The drawing under review shows one solid part. Ordinate dimensions are in mm from its lowest x, y, z. Coordinates: 2 decimals unless noted, no trailing zeros. Order: outer loops, then holes, each group sorted by start corner. A loop starts at its lowest first (then second) coordinate and runs counter-clockwise, first axis right, second up. Notation, with made-up numbers: (-30.5, 89.25) -> (23.5, 89.25) arc R22 cw to (23.5, 106.25) -> close; hole circle Ø1 at (17, -21). An arc over 180 degrees is marked (long way). Write item = value, one per line.
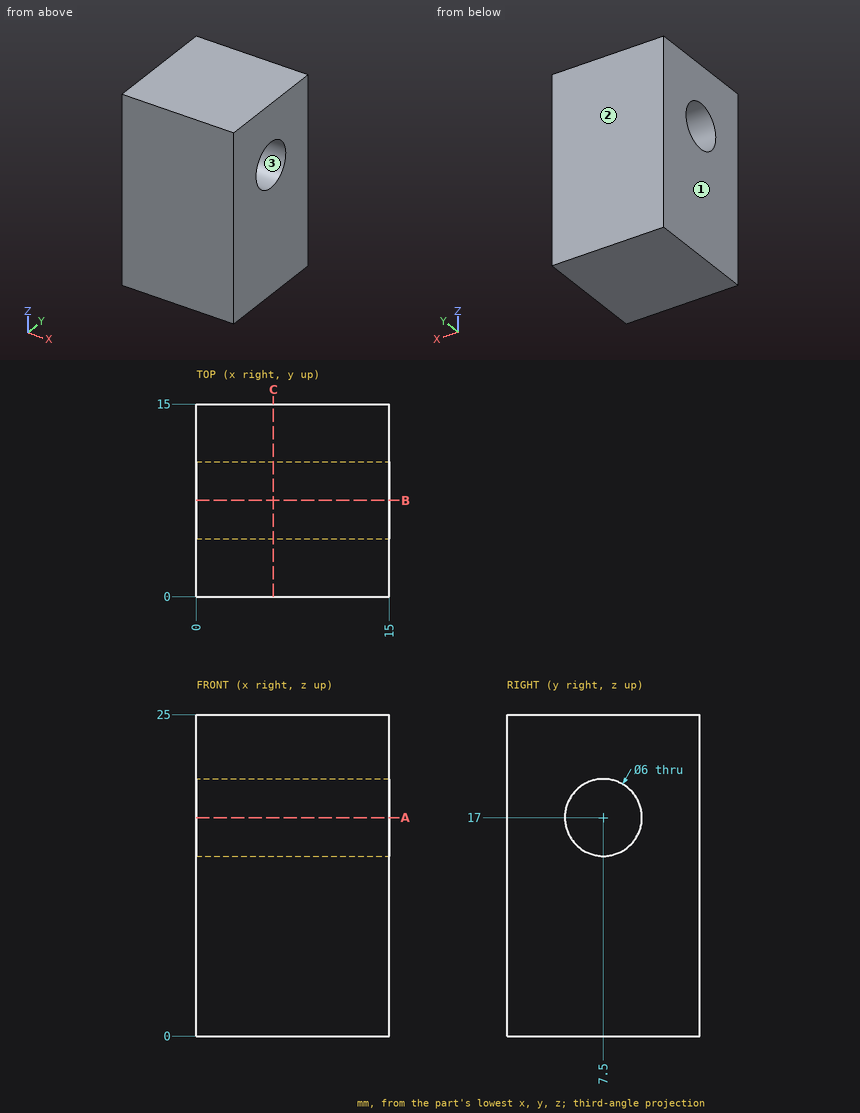
(1) We need section A-A (z = 17). Write out the cut boundary in (x, y), and give its area (3 significant figures).
Report:
outline = (0, 0) -> (15, 0) -> (15, 4.5) -> (0, 4.5) -> close; (0, 10.5) -> (15, 10.5) -> (15, 15) -> (0, 15) -> close
area = 135 mm²
(2) For L1, parallel to Y at x = 8, z = 17; L2, parallel to Z at x = 4, y = 7.5; L3, parallel to Y at x = 4, z = 14.5, list the stretches that pass through material, from the lowest coordinate up.
Report:
L1 = 0 to 4.5, 10.5 to 15
L2 = 0 to 14, 20 to 25
L3 = 0 to 5.84, 9.16 to 15
(3) The part is to be moulded in two halves that separate along Y. For the marked faces 1, 2 and 3, say which applies: released by +Y, released by -Y, zero draft, split by the parting line, or undercut.
Report:
face_1 = zero draft
face_2 = released by +Y
face_3 = undercut
(4) We need section C-C (x = 6). Write out the cut boundary in (y, z), and give its area (3 significant figures).
Report:
outline = (0, 0) -> (15, 0) -> (15, 25) -> (0, 25) -> close; hole circle Ø6 at (7.5, 17)
area = 347 mm²
(5) We need section B-B (y = 7.5). Write out the cut boundary in (x, z).
Report:
outline = (0, 0) -> (15, 0) -> (15, 14) -> (0, 14) -> close; (0, 20) -> (15, 20) -> (15, 25) -> (0, 25) -> close
